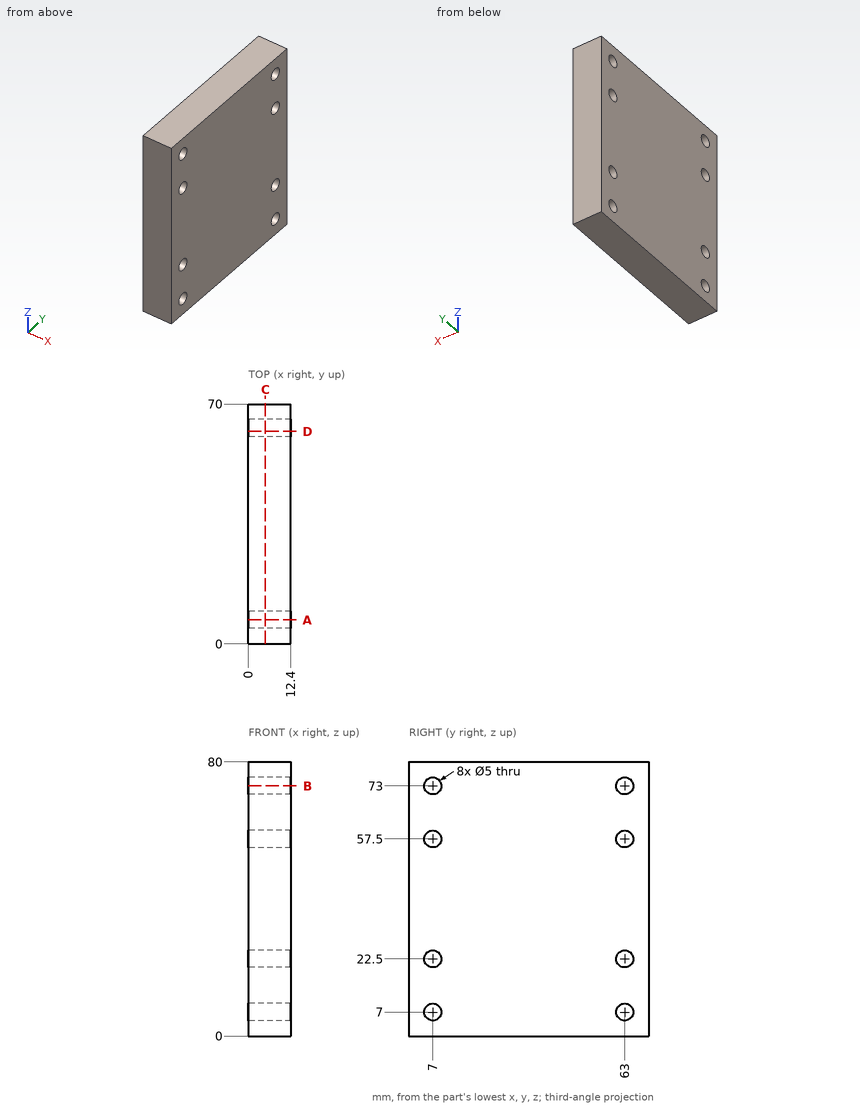
The figure shows three views and two pictorial views of one solid part (mm, origin at its lowest corner). Answer the questions. Coordinates: 2 decimals unless noted, no trailing zeros. Order: outer loops, then holes, each group sorted by start corner. A loop starts at its lowest first (then second) coordinate and runs counter-clockwise, first axis right, second up. Notation, with made-up numbers: (-12, -29.75) - (40, -29.75) arc R8 cw to (40, -20.75) - close; hole circle Ø1 at (57.25, 31). An arc over 180 degrees is marked (long way). Answer as a JSON object with one key per item and string values.
1. Find section B-B on z = 73. Determine the outline of the cut face in (x, y), plus the area to 3 significant figures.
Output values:
{"outline": "(0, 0) - (12.4, 0) - (12.4, 4.5) - (0, 4.5) - close; (0, 9.5) - (12.4, 9.5) - (12.4, 60.5) - (0, 60.5) - close; (0, 65.5) - (12.4, 65.5) - (12.4, 70) - (0, 70) - close", "area": "744 mm²"}
2. Find section C-C on x = 5. Count the separate pieces of the cut face and the enclosed holes in it, plus the area to 3 significant figures.
Output values:
{"separate pieces": "1", "enclosed holes": "8", "area": "5,440 mm²"}
3. Find section A-A on y = 7. Determine the outline of the cut face in (x, z).
Output values:
{"outline": "(0, 0) - (12.4, 0) - (12.4, 4.5) - (0, 4.5) - close; (0, 9.5) - (12.4, 9.5) - (12.4, 20) - (0, 20) - close; (0, 25) - (12.4, 25) - (12.4, 55) - (0, 55) - close; (0, 60) - (12.4, 60) - (12.4, 70.5) - (0, 70.5) - close; (0, 75.5) - (12.4, 75.5) - (12.4, 80) - (0, 80) - close"}
4. Find section D-D on y = 62. Determine the outline of the cut face in (x, z), plus the area to 3 significant figures.
Output values:
{"outline": "(0, 0) - (12.4, 0) - (12.4, 4.71) - (0, 4.71) - close; (0, 9.29) - (12.4, 9.29) - (12.4, 20.21) - (0, 20.21) - close; (0, 24.79) - (12.4, 24.79) - (12.4, 55.21) - (0, 55.21) - close; (0, 59.79) - (12.4, 59.79) - (12.4, 70.71) - (0, 70.71) - close; (0, 75.29) - (12.4, 75.29) - (12.4, 80) - (0, 80) - close", "area": "765 mm²"}
5. Consider line 1 (Y direction, x = 4.75, z = 73); line 2 (Z direction, x = 3.5, y = 64.5); line 3 (Y direction, x = 5, z = 6.5). Determine where each line is inside the solid, lowest interval first.
Output values:
{"line 1": "y = 0 to 4.5, 9.5 to 60.5, 65.5 to 70", "line 2": "z = 0 to 5, 9 to 20.5, 24.5 to 55.5, 59.5 to 71, 75 to 80", "line 3": "y = 0 to 4.55, 9.45 to 60.55, 65.45 to 70"}
